from build123d import *

# Parameters (mm, degrees)
SKETCH_1_W          = 50
SKETCH_1_H          = 40
EXTRUDE_1_DEPTH     = 20
SKETCH_2_R          = 10
CUT_EXTRUDE_1_DEPTH = 38.749172176
SKETCH_3_W          = 10
SKETCH_3_H          = 28
CUT_EXTRUDE_2_DEPTH = 38.749172176


with BuildPart() as part:
    # 草图1 → 凸台-拉伸1 (new body)
    with BuildSketch(Plane.XY):
        Rectangle(SKETCH_1_W, SKETCH_1_H)
    extrude(amount=EXTRUDE_1_DEPTH)

    # 草图2 → 切除-拉伸1 (cut, through all)
    with BuildSketch(Plane.XY.offset(20)):
        with Locations((0, 2.5)):
            Circle(SKETCH_2_R)
    extrude(amount=-CUT_EXTRUDE_1_DEPTH, mode=Mode.SUBTRACT)

    # 草图3 → 切除-拉伸2 (cut, through all)
    with BuildSketch(Plane.XY.offset(20)):
        with Locations((-20, 6)):
            Rectangle(SKETCH_3_W, SKETCH_3_H)
        with Locations((20, 6)):
            Rectangle(SKETCH_3_W, SKETCH_3_H)
    extrude(amount=-CUT_EXTRUDE_2_DEPTH, mode=Mode.SUBTRACT)


solid = part.part
Could you check a few things on this model? Use its own coordinates, in mm. A direction names the side the tool comes from. Round coordinates to 2 decimals unless told otherwise and drop trailing zeros. Write each loop counter-clockwise with the first axis right and the second up, starting at its lowest first coordinate (ties: lowest second). Pieces come first, ordered by that corner, then holes. Notation, with made-up numbers: (46.5, 53.25) - (105.5, 53.25) arc R24 cw to (105.5, 81.25) - close; hole circle Ø4 at (84.5, -17.75). An arc over 180 degrees is marked (long way). Put each result on its own line as item: value. Start each with the question number.
(1) I want a section at A-A, the plane y = 2.5. Please give me the cut outline in (x, z), plus the area to 3 significant figures.
(2) Thinking about a two-plate mould opening in X: for faces 4 (the cylindrical face through (5.38, 10.93, 10.14)), 5 (the flat face through (-25, -14, 10)), 6 (the flat face through (0, -9, 20)), which applies, released by +X, released by -X, zero draft, split by the parting line, or undercut?
(3) I need wall thicknesses on probe 1 along Y at (x, z) = (0, 6); probe 2 along X at (y, z) = (4, 1.75); probe 3 along X at (y, z) = (13, 15.5). Which ranges of each line are inside material? Lowest first, please.
(4) I want a section at C-C, the plane x = 0. Please give me the cut outline in (y, z), plus the area to 3 significant figures.
(5) I want a section at D-D, the plane x = -19.5. Please give me the cut outline in (y, z).
(6) I want a section at B-B, the plane z = 18.5. Please give me the cut outline in (x, y), plus the area to 3 significant figures.
(7) For faces 1 (the flat face through (-20, -8, 10)), 2 (the flat face through (20, -8, 10)), 3 (the flat face through (0, -20, 10)), which set-ups out of +Z, -Z, +X, -X, +Y, -Y let a thin tool reach every point of the face, with its end or its side?
(8) Will these pins go through, and if not, where does the flat tip stop? pin 1 (8 mm diameter, centred on x = 18, z = 10, fed in from +Y); pin 2 (6 mm diameter, centred on y = 3, z = 13.5, fed in from -X); pin 3 (3 mm diameter, centred on x = -17.5, z = 5.5, fed in from +Y); pin 4 (1.5 mm diameter, centred on y = 4, z = 12, fed in from +X).
Here are the results:
1. outline: (-15, 0) - (-10, 0) - (-10, 20) - (-15, 20) - close; (10, 0) - (15, 0) - (15, 20) - (10, 20) - close
1. area: 200 mm^2
2. face 4: undercut
2. face 5: released by -X
2. face 6: zero draft
3. probe 1: y = -20 to -7.5, 12.5 to 20
3. probe 2: x = -15 to -9.89, 9.89 to 15
3. probe 3: x = -15 to 15
4. outline: (-20, 0) - (-7.5, 0) - (-7.5, 20) - (-20, 20) - close; (12.5, 0) - (20, 0) - (20, 20) - (12.5, 20) - close
4. area: 400 mm^2
5. outline: (-20, 0) - (-8, 0) - (-8, 20) - (-20, 20) - close
6. outline: (-25, -20) - (25, -20) - (25, -8) - (15, -8) - (15, 20) - (-15, 20) - (-15, -8) - (-25, -8) - close; hole circle Ø20 at (0, 2.5)
6. area: 1,130 mm^2
7. face 1: +Z, -Z, -X, +Y
7. face 2: +Z, -Z, +X, +Y
7. face 3: +Z, -Z, +X, -X, -Y
8. pin 1: stops at y = 20
8. pin 2: stops at x = -15
8. pin 3: stops at y = -8
8. pin 4: stops at x = 15
